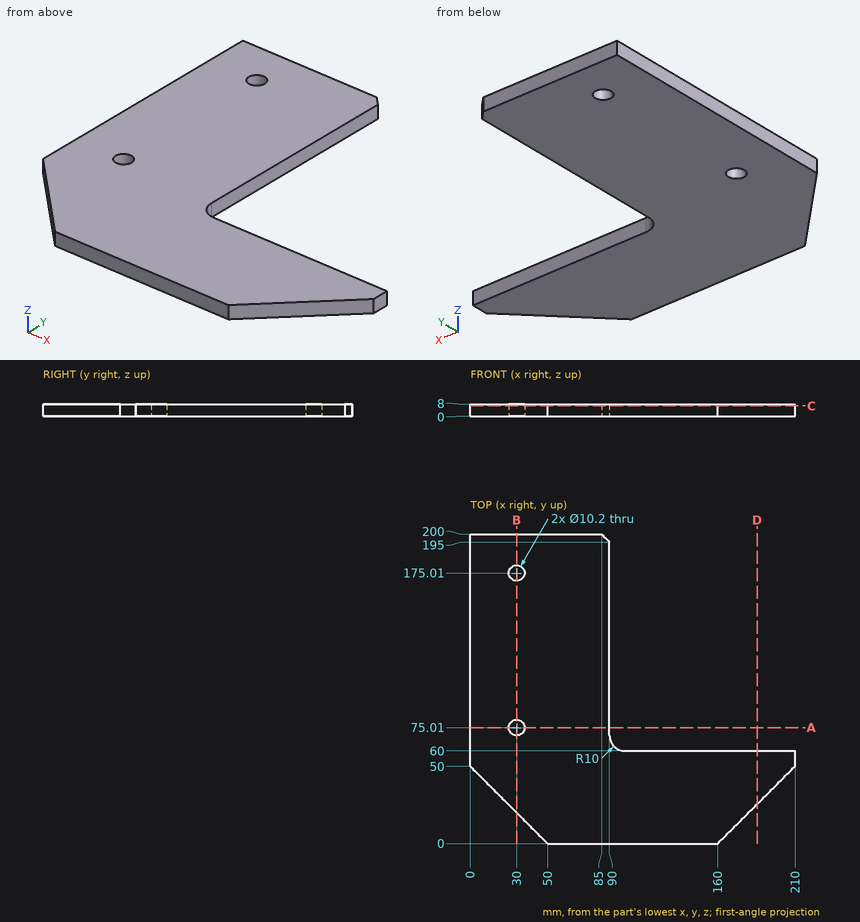
Geometry check sheet. Reference: drawing and pictorial views, mm from the part's lowest x, y, z. Round coordinates to 2 decimals unless told otherwise and drop trailing zeros. Write each loop counter-clockwise with the first axis right and the second up, starting at its lowest first coordinate (ties: lowest second). Pieces come first, ordered by that corner, then holes.
(1) Depth check by flat-ended pin: pin 1 Ø2.5 at (x, z) = (147, 2.5) entering from +Y; pin 2 Ø1 at (x, z) = (96, 5.5) entering from +Y; pin 3 Ø1 at (y, z) = (35, 3) entering from +X. Enter the tip coordinate at first touch or a pass-through.
Returned:
pin 1: stops at y = 60
pin 2: stops at y = 61.07
pin 3: stops at x = 195.5
(2) Section check C-C (z = 6.75). Enter the section's corners in (x, y).
Returned:
outline: (0, 50) - (50, 0) - (160, 0) - (210, 50) - (210, 60) - (100, 60) arc R10 cw to (90, 70) - (90, 195) - (85, 200) - (0, 200) - close; hole circle Ø10.2 at (30, 75.01); hole circle Ø10.2 at (30, 175.01)
(3) Section check B-B (x = 30). Enter the section's corners in (y, z).
Returned:
outline: (20, 0) - (69.91, 0) - (69.91, 8) - (20, 8) - close; (80.11, 0) - (169.91, 0) - (169.91, 8) - (80.11, 8) - close; (180.11, 0) - (200, 0) - (200, 8) - (180.11, 8) - close
(4) Section check A-A (y = 75.01). Enter the section's corners in (x, z), plus the area to 3 significant figures.
Returned:
outline: (0, 0) - (24.9, 0) - (24.9, 8) - (0, 8) - close; (35.1, 0) - (90, 0) - (90, 8) - (35.1, 8) - close
area: 638 mm2
(5) Material ranges on line 1 (Y direction, x = 30, z = 4.5); line 2 (X direction, y = 111, z = 0.5); line 3 (Y direction, x = 101, z = 7.75), recorded low to high.
Returned:
line 1: y = 20 to 69.91, 80.11 to 169.91, 180.11 to 200
line 2: x = 0 to 90
line 3: y = 0 to 60
(6) Section check D-D (x = 185.5). Enter the section's corners in (y, z).
Returned:
outline: (25.5, 0) - (60, 0) - (60, 8) - (25.5, 8) - close
